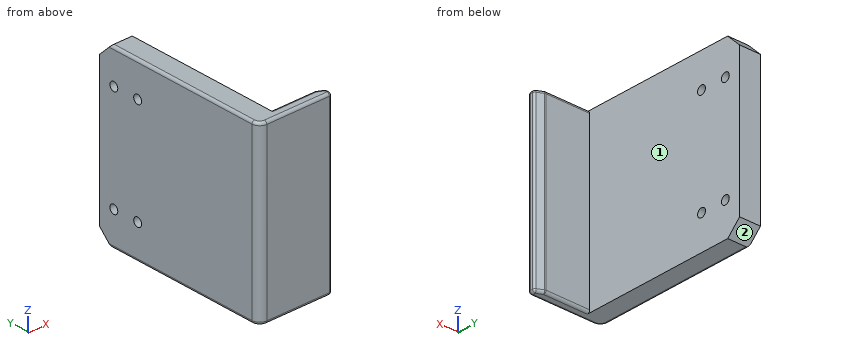
from build123d import *

# Parameters (mm, degrees)
EXTRUDE_1_DEPTH    = 33
CHAMFER_1_SIZE     = 1.5
CHAMFER_1_SIZE2    = 3
FILLET_1_R         = 1
CHAMFER_2_SIZE     = 5
FILLET_3_R         = 3
FILLET_4_R         = 1
HOLE_WIZARD_M4_2_D = 3.3


with BuildPart() as part:
    # 草图1 → 凸台-拉伸1 (new, symmetric)
    with BuildSketch(Plane.XY):
        Polygon((0, 67), (0, 0), (28, 0), (28, 4), (8, 4), (8, 67), align=None)
    extrude(amount=EXTRUDE_1_DEPTH, both=True)

    # 倒角1
    chamfer_1_edges = [part.edges().sort_by_distance(p)[0] for p in [
        (28, 4, 0),
    ]]
    chamfer_1_side = [part.faces().sort_by_distance(p)[0] for p in [
        (28, 2, 0),
    ]]
    chamfer(chamfer_1_edges, length=CHAMFER_1_SIZE, length2=CHAMFER_1_SIZE2, reference=chamfer_1_side[0])

    # 圆角1
    fillet_1_edges = [part.edges().sort_by_distance(p)[0] for p in [
        (28, 0, 0),
        (25, 4, 0),
        (28, 2.5, 0),
    ]]
    fillet(fillet_1_edges, radius=FILLET_1_R)

    # 倒角2
    chamfer_2_edges = [part.edges().sort_by_distance(p)[0] for p in [
        (4, 67, 33),
        (4, 67, -33),
    ]]
    chamfer(chamfer_2_edges, length=CHAMFER_2_SIZE)

    # 圆角3
    fillet_3_edges = [part.edges().sort_by_distance(p)[0] for p in [
        (0, 0, 0),
    ]]
    fillet(fillet_3_edges, radius=FILLET_3_R)

    # 圆角4
    fillet_4_edges = [part.edges().sort_by_distance(p)[0] for p in [
        (28, 1.440983006, -33),
        (28, 1.440983006, 33),
        (16.381966011, 4, -33),
        (26.329179607, 3.335410197, -33),
        (24.993684943, 3.973248989, -33),
        (27.850650808, 2.407697123, -33),
        (27.707106781, 0.292893219, -33),
        (26.329179607, 3.335410197, 33),
        (16.381966011, 4, 33),
        (24.993684943, 3.973248989, 33),
        (27.850650808, 2.407697123, 33),
        (27.707106781, 0.292893219, 33),
        (0, 32.5, 33),
        (0, 32.5, -33),
        (15, 0, -33),
        (15, 0, 33),
        (0.878679656, 0.878679656, -33),
        (0.878679656, 0.878679656, 33),
    ]]
    fillet(fillet_4_edges, radius=FILLET_4_R)

    # M4 螺纹孔2 (through all)
    with Locations(Plane.ZY):
        with Locations((-20, 61), (20, 61), (-20, 51), (20, 51)):
            Hole(HOLE_WIZARD_M4_2_D / 2)


solid = part.part
Read the model definition and answer for the solid it produces. Units are mm, in the model's axes. Face numbers are marked on the shaded views. A direction names the side the tool comes from. Round coordinates to 2 decimals unless told otherwise and drop trailing zeros. Write each loop counter-clockwise with the first axis right and the second up, starting at its lowest first coordinate (ties: lowest second). Pieces come first, ordered by that corner, then holes.
1. The part is cut by section D-D, the plane x = 21.75. Determine the outline of the cut face in (y, z), then the cut area to 3 significant figures.
2. Straight lines are drawn through the part: L1, parallel to Y at x = 3.75, z = -20; L2, parallel to X at y = 50.5, z = -14; L3, parallel to Y at x = 19, z = 16. For each, find the intervals that lie inside material, in ascending order.
3. The part is cut by section C-C, the plane z = 17.5. Determine the outline of the cut face in (x, y).
4. The part is cut by section A-A, the plane z = -20. Determine the outline of the cut face in (x, y), then the cut area to 3 significant figures.
5. Which of the six approach directions +Z, -Z, +X, -X, +Y, -Y give full straight-line access (tool end or side, diameter ignored) to the marked faces 1 and 2?
6. The part is cut by section B-B, the plane y = 51. Determine the outline of the cut face in (x, z), then the cut area to 3 significant figures.
7. Given pin 1 Ø5.5 at (y, z) = (61, 20) entering from +X; pin 2 Ø6 at (x, z) = (20.5, -22) entering from +Y, each flat-ended and moving along its own axis, determine where each tip first touches the part or whether it passes through.
Values:
1. outline: (0, -32) arc R1 ccw to (1, -33) - (3, -33) arc R1 ccw to (4, -32) - (4, 32) arc R1 ccw to (3, 33) - (1, 33) arc R1 ccw to (0, 32) - close
1. area: 263 mm2
2. L1: y = 0 to 49.35, 52.65 to 59.35, 62.65 to 67
2. L2: x = 0 to 8
2. L3: y = 0 to 4
3. outline: (0, 3) arc R3 ccw to (3, 0) - (27, 0) arc R1 ccw to (28, 1) - (28, 1.88) arc R1 ccw to (27.45, 2.78) - (25.21, 3.89) arc R1 ccw to (24.76, 4) - (8, 4) - (8, 67) - (0, 67) - close
4. outline: (0, 3) arc R3 ccw to (3, 0) - (27, 0) arc R1 ccw to (28, 1) - (28, 1.88) arc R1 ccw to (27.45, 2.78) - (25.21, 3.89) arc R1 ccw to (24.76, 4) - (8, 4) - (8, 49.35) - (0, 49.35) - close; (0, 52.65) - (8, 52.65) - (8, 59.35) - (0, 59.35) - close; (0, 62.65) - (8, 62.65) - (8, 67) - (0, 67) - close
4. area: 559 mm2
5. face 1: +Z, -Z, +X, +Y
5. face 2: -Z, +X, -X, +Y
6. outline: (0, -32) arc R1 ccw to (1, -33) - (8, -33) - (8, -21.65) - (0, -21.65) - close; (0, -18.35) - (8, -18.35) - (8, 18.35) - (0, 18.35) - close; (0, 21.65) - (8, 21.65) - (8, 33) - (1, 33) arc R1 ccw to (0, 32) - close
6. area: 475 mm2
7. pin 1: stops at x = 8
7. pin 2: stops at y = 4
